Check sheet for the modelled part. Datum: model origin and axes. Units: mm. Face numbers are marked on the shaded views. A direction names the side the tool comes from. Coordinates: 2 decimals unless noted, no trailing zeros. Write each loop counter-clockwise with the first axis right and the second up, starting at its lowest first coordinate (ties: lowest second). Pieces come first, ordered by that corner, then holes. Notation, with made-up numbers: (-37.5, 40) - (6.5, 40) arc R33 cw to (6.5, 76) - close; hole circle Ø9 at (68.25, -29.75). An arc over 180 degrees is marked (long way). Use one line per item in the form item = value. Start each with the question number.
1. Go/stop test with flat-tipped pins: pin 1 Ø6.5 at (y, z) = (14.5, -195) entering from +X; pin 2 Ø9 at (y, z) = (30.5, -195) entering from +X; pin 3 Ø23 at (x, z) = (22, -27.5) entering from +Y; pin 4 Ø4.5 at (y, z) = (14.5, -185) entering from +X. Record where each tip stops, or that it passes through.
2. Cross-section at B-B on x = 11. Record the boundary of the cut face in (y, z).
3. Tool access check on the marked faces 1 and 2. Record the directions out of +Z, -Z, +X, -X, +Y, -Y that give a thin tool (end or side, any length) a straight path to the whole face; none if there is none.
4. Cross-section at A-A on z = -63.5. Record the boundary of the cut face in (x, y).
5. Scan lines: line 1 along Y through (x, z) = (0.85, 185); line 2 along Z through (x, y) = (0.65, 30.5); line 3 along Y through (x, z) = (38, 249). Record each from-to range of solid material in increasing order.
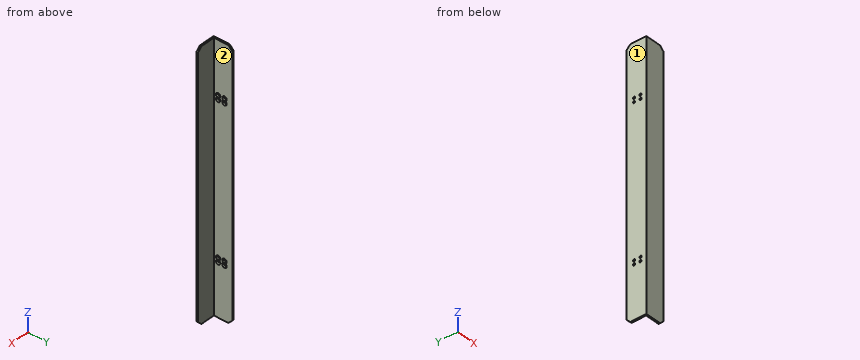
```python
from build123d import *

# Parameters (mm, degrees)
EXTRUDE_1_DEPTH             = 325
CHAMFER_1_SIZE              = 10
HOLE_WIZARD_M5_2_AT_2_COUNT = 2
HOLE_WIZARD_M5_2_AT_2_PITCH = 380
HOLE_WIZARD_M5_2_AT_3_COUNT = 2
HOLE_WIZARD_M5_2_AT_3_PITCH = 10
HOLE_WIZARD_M5_2_AT_4_COUNT = 2
HOLE_WIZARD_M5_2_AT_4_PITCH = 390
HOLE_WIZARD_M5_2_AT_5_COUNT = 2
HOLE_WIZARD_M5_2_AT_5_PITCH = 16
HOLE_WIZARD_M5_2_AT_6_COUNT = 2
HOLE_WIZARD_M5_2_AT_6_PITCH = 380.336692945
HOLE_WIZARD_M5_2_AT_7_COUNT = 2
HOLE_WIZARD_M5_2_AT_7_PITCH = 18.867962264
HOLE_WIZARD_M5_2_AT_8_COUNT = 2
HOLE_WIZARD_M5_2_AT_8_PITCH = 390.328067144


with BuildPart() as part:
    # 草图1 → 凸台-拉伸1 (new, symmetric)
    with BuildSketch(Plane.XY):
        Polygon((0, 0), (50, 0), (50, 4), (4, 4), (4, 50), (0, 50), align=None)
    extrude(amount=EXTRUDE_1_DEPTH, both=True)

    # 倒角1
    chamfer_1_edges = [part.edges().sort_by_distance(p)[0] for p in [
        (50, 2, 325),
        (2, 50, 325),
        (2, 50, -325),
        (50, 2, -325),
    ]]
    chamfer(chamfer_1_edges, length=CHAMFER_1_SIZE)

    # 草图5 → M5 六角凹锥坑螺钉的锥形沉头孔2 (revolve, cut)
    with BuildSketch(Plane(origin=(4, 30.5, 195), x_dir=(0, 0, -1), z_dir=(0, 1, 0))):
        Polygon((0, 0), (0, 4), (2.75, 4), (2.75, 2.85), (5.6, 0), align=None)
    hole_wizard_m5_2 = revolve(axis=Axis((10.35, 30.5, 195), (-1, 0, 0)), mode=Mode.SUBTRACT)

    # M5 六角凹锥坑螺钉的锥形沉头孔2 at 2: M5 六角凹锥坑螺钉的锥形沉头孔2 ×2
    with Locations(*[(0, 0, -i * HOLE_WIZARD_M5_2_AT_2_PITCH) for i in range(1, HOLE_WIZARD_M5_2_AT_2_COUNT)]):
        add(hole_wizard_m5_2, mode=Mode.SUBTRACT)

    # M5 六角凹锥坑螺钉的锥形沉头孔2 at 3: M5 六角凹锥坑螺钉的锥形沉头孔2 ×2
    with Locations(*[(0, 0, -i * HOLE_WIZARD_M5_2_AT_3_PITCH) for i in range(1, HOLE_WIZARD_M5_2_AT_3_COUNT)]):
        add(hole_wizard_m5_2, mode=Mode.SUBTRACT)

    # M5 六角凹锥坑螺钉的锥形沉头孔2 at 4: M5 六角凹锥坑螺钉的锥形沉头孔2 ×2
    with Locations(*[(0, 0, -i * HOLE_WIZARD_M5_2_AT_4_PITCH) for i in range(1, HOLE_WIZARD_M5_2_AT_4_COUNT)]):
        add(hole_wizard_m5_2, mode=Mode.SUBTRACT)

    # M5 六角凹锥坑螺钉的锥形沉头孔2 at 5: M5 六角凹锥坑螺钉的锥形沉头孔2 ×2
    with Locations(*[(0, -i * HOLE_WIZARD_M5_2_AT_5_PITCH, 0) for i in range(1, HOLE_WIZARD_M5_2_AT_5_COUNT)]):
        add(hole_wizard_m5_2, mode=Mode.SUBTRACT)

    # M5 六角凹锥坑螺钉的锥形沉头孔2 at 6: M5 六角凹锥坑螺钉的锥形沉头孔2 ×2
    with Locations(*[Vector(0, -0.04206798948618002, -0.9991147502967769) * (i * HOLE_WIZARD_M5_2_AT_6_PITCH) for i in range(1, HOLE_WIZARD_M5_2_AT_6_COUNT)]):
        add(hole_wizard_m5_2, mode=Mode.SUBTRACT)

    # M5 六角凹锥坑螺钉的锥形沉头孔2 at 7: M5 六角凹锥坑螺钉的锥形沉头孔2 ×2
    with Locations(*[Vector(0, -0.8479983040050839, -0.5299989400031865) * (i * HOLE_WIZARD_M5_2_AT_7_PITCH) for i in range(1, HOLE_WIZARD_M5_2_AT_7_COUNT)]):
        add(hole_wizard_m5_2, mode=Mode.SUBTRACT)

    # M5 六角凹锥坑螺钉的锥形沉头孔2 at 8: M5 六角凹锥坑螺钉的锥形沉头孔2 ×2
    with Locations(*[Vector(0, -0.04099115935241401, -0.9991595092150928) * (i * HOLE_WIZARD_M5_2_AT_8_PITCH) for i in range(1, HOLE_WIZARD_M5_2_AT_8_COUNT)]):
        add(hole_wizard_m5_2, mode=Mode.SUBTRACT)


solid = part.part
```
Final values:
q1.pin_1 = 1.65
q1.pin_2 = 2.9
q1.pin_3 = 4
q1.pin_4 = through
q2.outline = (0, -325) - (4, -325) - (4, 325) - (0, 325) - close
q3.face_1 = +Z, -Z, -X, +Y, -Y
q3.face_2 = +Z, -Z, +X, +Y
q4.outline = (0, 0) - (50, 0) - (50, 4) - (4, 4) - (4, 50) - (0, 50) - close
q5.line_1 = 0 to 11.75, 17.25 to 27.75, 33.25 to 50
q5.line_2 = -325 to -197.75, -192.25 to -187.75, -182.25 to 182.25, 187.75 to 192.25, 197.75 to 325
q5.line_3 = 0 to 4
